```python
from build123d import *

# Parameters (mm, degrees)
EXTRUDE_1_DEPTH          = 2005
EXTRUDE_1_2_DEPTH        = 28
SKETCH_5_W               = 2
SKETCH_5_H               = 139.764501988
EXTRUDE_2_DEPTH          = 28
SKETCH_6_W               = 269.171572875
SKETCH_6_H               = 2
EXTRUDE_3_DEPTH          = 28
SKETCH_7_W               = 2
SKETCH_7_H               = 2005
EXTRUDE_4_DEPTH          = 28
CUT_EXTRUDE_1_DEPTH      = 10
CUT_EXTRUDE_1_DEPTH_BACK = 10
SKETCH_8_R               = 4.5
SKETCH_9_R               = 4.5
CUT_EXTRUDE_2_DEPTH      = 10
SKETCH_10_R              = 4.5
CUT_EXTRUDE_3_DEPTH      = 76
SKETCH_11_R              = 4.5
CUT_EXTRUDE_4_DEPTH      = 63
SKETCH_12_R              = 4.5
CUT_EXTRUDE_5_DEPTH      = 10
SKETCH_13_R              = 4.5
CUT_EXTRUDE_6_DEPTH      = 10


with BuildPart() as part:
    # 草图1 → Extrude 1 (new body)
    with BuildSketch(Plane.XY):
        Polygon((0, 0), (270, 0), (370, 100), (370, 270), (368, 270), (368, 100.828427125), (269.171572875, 2), (0, 2), align=None)
    extrude(amount=EXTRUDE_1_DEPTH)

    # 草图4 → Extrude 1 2 (add)
    with BuildSketch(Plane.ZY.offset(-368)):
        Polygon((0, 100.828427125), (0, 270), (2005, 270), (2005, 100.828427125), (2003, 100.828427125), (2003, 268), (2, 268), (2, 100.828427125), align=None)
    extrude(amount=EXTRUDE_1_2_DEPTH)

    # 草图5 → 凸台-拉伸2 (add)
    with BuildSketch(Plane(origin=(133.585786438, -133.585786438, 0), x_dir=(0, 0, 1), z_dir=(-0.7071067811865476, 0.7071067811865476, 0))):
        with Locations((1, 261.629509039)):
            Rectangle(SKETCH_5_W, SKETCH_5_H)
        with Locations((2004, 261.629509039)):
            Rectangle(SKETCH_5_W, SKETCH_5_H)
    extrude(amount=EXTRUDE_2_DEPTH)

    # 草图6 → 凸台-拉伸3 (add)
    with BuildSketch(Plane(origin=(0, 2, 0), x_dir=(1, 0, 0), z_dir=(0, 1, 0))):
        with Locations((134.585786438, -1)):
            Rectangle(SKETCH_6_W, SKETCH_6_H)
        with Locations((134.585786438, -2004)):
            Rectangle(SKETCH_6_W, SKETCH_6_H)
    extrude(amount=EXTRUDE_3_DEPTH)

    # 草图7 → 凸台-拉伸4 (add)
    with BuildSketch(Plane(origin=(0, 2, 0), x_dir=(1, 0, 0), z_dir=(0, 1, 0))):
        with Locations((1, -1002.5)):
            Rectangle(SKETCH_7_W, SKETCH_7_H)
    extrude(amount=EXTRUDE_4_DEPTH)

    # 草图8 → 切除-拉伸1 (cut, two sides: drawn at the far end of the back side and taken through both)
    with BuildSketch(Plane(origin=(0, 0, 2003), x_dir=(-1, 0, 0), z_dir=(0, 0, -1)).offset(-CUT_EXTRUDE_1_DEPTH_BACK)):
        with Locations(Location((-354, 240, 0), (0, 0, 180))):
            Circle(SKETCH_8_R)
        with Locations(Location((-30, 16, 0), (0, 0, 180))):
            Circle(SKETCH_8_R)
        with Locations(Location((-354, 140, 0), (0, 0, 180))):
            Circle(SKETCH_8_R)
        with Locations(Location((-160, 16, 0), (0, 0, 180))):
            Circle(SKETCH_8_R)
    extrude(amount=CUT_EXTRUDE_1_DEPTH + CUT_EXTRUDE_1_DEPTH_BACK, mode=Mode.SUBTRACT)

    # 草图9 → 切除-拉伸2 (cut)
    with BuildSketch(Plane.XZ.offset(-268)):
        with Locations(Location((354, 1975, 0), (0, 0, 270))):
            Circle(SKETCH_9_R)
        with Locations(Location((354, 1825, 0), (0, 0, 270))):
            Circle(SKETCH_9_R)
    extrude(amount=-CUT_EXTRUDE_2_DEPTH, mode=Mode.SUBTRACT)

    # 草图10 → 切除-拉伸3 (cut)
    with BuildSketch(Plane(origin=(2, 0, 0), x_dir=(0, 0, -1), z_dir=(1, 0, 0))):
        with Locations((-1975, 16)):
            Circle(SKETCH_10_R)
        with Locations((-1825, 16)):
            Circle(SKETCH_10_R)
    extrude(amount=-CUT_EXTRUDE_3_DEPTH, mode=Mode.SUBTRACT)

    # 草图11 → 切除-拉伸4 (cut)
    with BuildSketch(Plane.XZ.offset(-268)):
        with Locations(Location((354, 30, 0), (0, 0, 270))):
            Circle(SKETCH_11_R)
        with Locations(Location((354, 210, 0), (0, 0, 270))):
            Circle(SKETCH_11_R)
    extrude(amount=-CUT_EXTRUDE_4_DEPTH, mode=Mode.SUBTRACT)

    # 草图12 → 切除-拉伸5 (cut)
    with BuildSketch(Plane(origin=(2, 0, 0), x_dir=(0, 0, -1), z_dir=(1, 0, 0))):
        with Locations((-30, 16)):
            Circle(SKETCH_12_R)
        with Locations((-442, 16)):
            Circle(SKETCH_12_R)
    extrude(amount=-CUT_EXTRUDE_5_DEPTH, mode=Mode.SUBTRACT)

    # 草图13 → 切除-拉伸6 (cut)
    with BuildSketch(Plane(origin=(0, 0, 0), x_dir=(-1, 0, 0), z_dir=(0, 0, -1))):
        with Locations(Location((-30, 16, 0), (0, 0, 180))):
            Circle(SKETCH_13_R)
        with Locations(Location((-354, 240, 0), (0, 0, 180))):
            Circle(SKETCH_13_R)
        with Locations((-308.686291501, 61.313708499)):
            Circle(SKETCH_13_R)
    extrude(amount=-CUT_EXTRUDE_6_DEPTH, mode=Mode.SUBTRACT)


solid = part.part
```
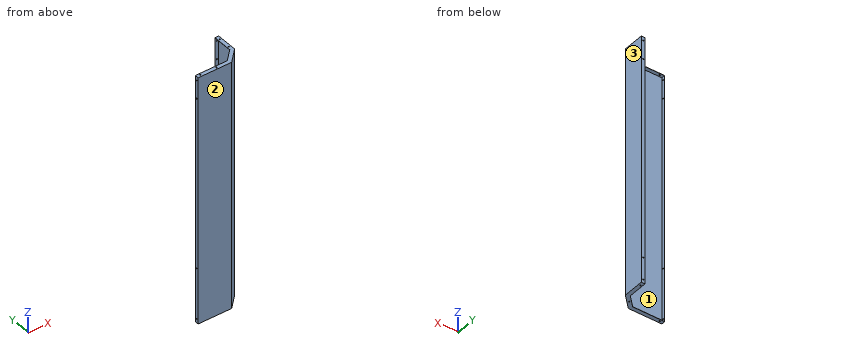
The listing builds one solid part. Answer for the finished solid, in the listing's coordinates (mm). Face numbers are marked on the shaded views. Coordinates: 2 decimals unless noted, no trailing zeros. Loops run counter-clockwise (first coordinate to the right, second up) from the corner with the lowest first, then second, coordinate; pieces in that order, holes last. Notation, with made-up numbers: M -34.5,71 L -9.5,71 A25 ccw -9.5,92 Z; hole C 17.25,3.5 d2. An arc over 180 degrees is marked long. Answer as a JSON object with one key per item and string values. Group by question number.
Item 1: Each of these flat-tipped pins is pushed along its axis until it touches: P1, Ø5.5, axis at y = 16, z = 1825, coming from the -X side; P2, Ø10.5, axis at x = 354, z = 1975, coming from the -Y side; P3, Ø8.5, axis at x = 360.5, z = 1384, coming from the -Y side; P4, Ø2, axis at x = 131, y = 31.5, coming from the +Z side. Where does it stop, or does it pass through?
Item 2: Consider L1, parallel to Z at x = 354, y = 269.1; L2, parallel to Y at x = 160, z = 2003.7; L3, parallel to X at y = 254.5, z = 1037.5. Determine where each line is inside the solid, lowest interval first.
Item 3: Determine the mould class of the marked faces 1, 2 and 3 for opening direction X: +X half, -X half, draft (parallel to the pull), parting line (faces both ways), or undercut.
Item 4: Section A-A (x = 75.5) is taken. Write down the section's boundary in (y, z).
Item 5: Section B-B (z = 584.5) is taken. Write down the section's boundary in (x, y).
Solved:
{
 "1": {"P1": "stops at x = 280.42", "P2": "stops at y = 78.75", "P3": "stops at y = 86.25", "P4": "passes through"},
 "2": {"L1": "z = 0 to 25.5, 34.5 to 205.5, 214.5 to 1820.5, 1829.5 to 1970.5, 1979.5 to 2005", "L2": "y = 0 to 11.5, 20.5 to 30", "L3": "x = 368 to 370"},
 "3": {"face 1": "undercut", "face 2": "draft", "face 3": "+X half"},
 "4": {"outline": "M 0,0 L 30,0 L 30,2 L 2,2 L 2,2003 L 30,2003 L 30,2005 L 0,2005 Z"},
 "5": {"outline": "M 0,0 L 270,0 L 370,100 L 370,270 L 340,270 L 340,268 L 368,268 L 368,100.83 L 269.17,2 L 2,2 L 2,30 L 0,30 Z"}
}
